The listing builds one solid part. Answer for the finished solid, in the listing's coordinates (mm). A direction names the side the tool comes from. Round coordinates to 2 decimals unless told otherwise and drop trailing zeros. Order: outer loops, then holes, each group sorted by start corner. A loop starts at its lowest first (then second) coordinate and runs counter-clockwise, first axis right, second up. Notation, with made-up numbers: (-29.75, -10.5) -> (27.25, -10.5) arc R18 ccw to (27.25, -4.5) -> close; hole circle Ø7 at (55.5, 78). An arc over 180 degrees is marked (long way). Answer in a Markdown table with one row per item. Add a question column.
```python
from build123d import *

# Parameters (mm, degrees)
BASE_WEDGE_BLOCK_DEPTH = 87.5
TWIN_START             = -200
TWIN_SLOTS_15MM_DEPTH  = 200


with BuildPart() as part:
    # Base Profile Sketch → Base Wedge Block (new, symmetric)
    with BuildSketch(Plane.XY):
        Polygon((-96.311034199, 0), (103.688965801, 0), (103.688965801, 50), (75, 50), (0, 125), (-75, 50), (-96.311034199, 50), align=None)
    extrude(amount=BASE_WEDGE_BLOCK_DEPTH, both=True)

    # Slot Profile Sketch → Twin Slots 15mm (add)
    with BuildSketch(Plane(origin=(103.688965801, 0, 0), x_dir=(0, 0, -1), z_dir=(1, 0, 0)).offset(TWIN_START)):
        Polygon((-87.5, 0), (-87.5, 50), (-37.5, 50), (-37.5, 100), (-22.5, 100), (-22.5, 65), (22.5, 65), (22.5, 100), (37.5, 100), (37.5, 50), (87.5, 50), (87.5, 0), align=None)
    extrude(amount=TWIN_SLOTS_15MM_DEPTH)


solid = part.part
```
Item 1: The part is cut by section A-A, the plane x = 50. Give the vertices of the cut face in (y, z).
Item 2: The part is cut by section B-B, the plane y = 97.5. Give the vertices of the cut face in (x, z), and give its area (3 significant figures).
Item 3: For a pull along Z with two mould halves and no side action, classify faces 1 (the face through (-69, 80, 37.5)), 2 (the face through (73, 82, -22.5)), 3 (the face through (90, 50, 63)) as released by +Z, released by -Z, zero draft, split by the parting line, or undercut.
Item 4: Flat-ended cylindrical pins translate along their axes: P1, Ø16.5, axis at x = -59.5, z = -32.5, coming from the +Y side; P2, Ø6, axis at x = 4.5, z = -50, coming from the +Y side; P3, Ø1, axis at x = -30, z = 65.5, coming from the +Y side. Find the tip coordinate at first contact, or state that the pin passes through.
Item 5: The part is cut by section D-D, the plane x = 70. Give the vertices of the cut face in (y, z).
Item 6: Find the intervals of material crossed by probe 1 along Y at (x, z) = (-74, -22); probe 2 along Y at (x, z) = (-86, -75); probe 3 along X at (y, z) = (80, 13), in increasing order. Write a range as [from, to].
Item 7: A tool of negligible diameter and unlimited length cuts with its end or side. For faces 4 (the face through (-69, 81, -37.5)), 5 (the face through (64, 100, -30)), 6 (the face through (-69, 82, -22.5)), from which of +Z, -Z, +X, -X, +Y, -Y can it reach the whole face along a straight path? Write none if from no direction.
Item 8: The part is cut by section C-C, the plane z = 18.5. Give the vertices of the cut face in (x, y), and give its area (3 significant figures).
Resolved:
| question | item | result |
|---|---|---|
| 1 | outline | (0, -87.5) -> (75, -87.5) -> (75, -37.5) -> (100, -37.5) -> (100, -22.5) -> (75, -22.5) -> (75, 22.5) -> (100, 22.5) -> (100, 37.5) -> (75, 37.5) -> (75, 87.5) -> (0, 87.5) -> close |
| 2 | outline | (-96.31, -37.5) -> (-27.5, -37.5) -> (-27.5, -87.5) -> (27.5, -87.5) -> (27.5, -37.5) -> (103.69, -37.5) -> (103.69, -22.5) -> (27.5, -22.5) -> (27.5, 22.5) -> (103.69, 22.5) -> (103.69, 37.5) -> (27.5, 37.5) -> (27.5, 87.5) -> (-27.5, 87.5) -> (-27.5, 37.5) -> (-96.31, 37.5) -> (-96.31, 22.5) -> (-27.5, 22.5) -> (-27.5, -22.5) -> (-96.31, -22.5) -> close |
| 2 | area | 14,000 mm2 |
| 3 | face 1 | released by +Z |
| 3 | face 2 | undercut |
| 3 | face 3 | zero draft |
| 4 | P1 | y = 100 |
| 4 | P2 | y = 123.5 |
| 4 | P3 | y = 95.5 |
| 5 | outline | (0, -87.5) -> (55, -87.5) -> (55, -37.5) -> (100, -37.5) -> (100, -22.5) -> (65, -22.5) -> (65, 22.5) -> (100, 22.5) -> (100, 37.5) -> (55, 37.5) -> (55, 87.5) -> (0, 87.5) -> close |
| 6 | probe 1 | [0, 65] |
| 6 | probe 2 | [0, 50] |
| 6 | probe 3 | [-45, 45] |
| 7 | face 4 | -Z, -X, +Y |
| 7 | face 5 | +Z, -Z, +X, +Y |
| 7 | face 6 | -X, +Y |
| 8 | outline | (-96.31, 0) -> (103.69, 0) -> (103.69, 65) -> (60, 65) -> (0, 125) -> (-60, 65) -> (-96.31, 65) -> close |
| 8 | area | 16,600 mm2 |
